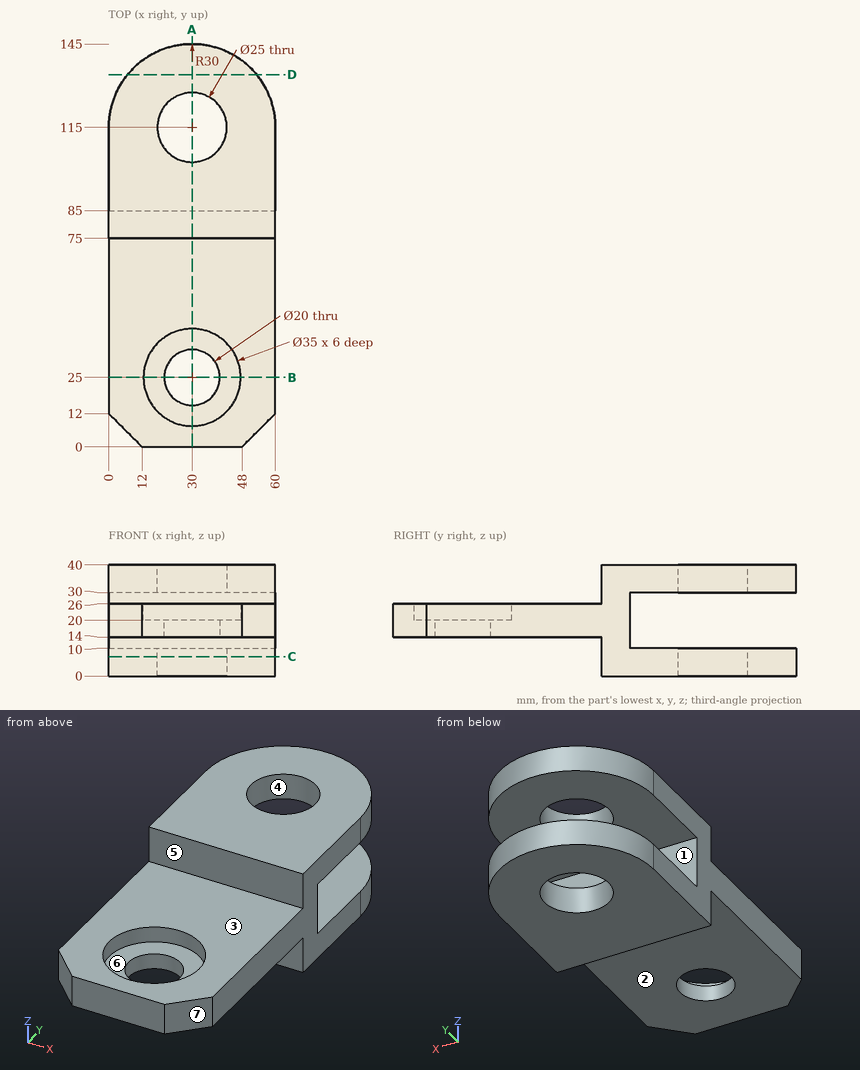
Design review of the part shown in the three views and the two pictorial views. Dimensions are in mm from the part's minimum x, y and z. A direction names the side the tool comes from. Give positions to 0.01 mm unless a question says otherwise; leave off trailing zeros. Loops run counter-clockwise (first coordinate to the right, second up) from the corner with the lowest first, then second, coordinate; pieces in that order, holes last. Notation, with made-up numbers: (19.5, 67) - (44.5, 67) arc R17 cw to (44.5, 79) - close; hole circle Ø9 at (-6, -9.5). An arc over 180 degrees is marked (long way). Use CSV: the item, a comma, the result in double quotes. Start each with the question number.
1. Wall thickness on L1, parallel to Z at x = 15, y = 127; L2, parallel to Y at x = 30, z = 7.75; L3, parallel to Y at x = 30, z = 18.6: over which ranges is each line inside the solid? List them lowest first.
2. Add section A-A (x = 30). State the section outline as (y, z) points, plus the area to 3 significant figures.
3. Insertion check: P1, Ø18, axis at x = 40.5, y = 52.5, coming from the -Z side; P2, Ø5, axis at y = 114, z = 13.5, coming from the -X side; P3, Ø4, axis at x = 31, z = 13, coming from the +Y side; P4, Ø10, axis at x = 36.5, y = 40, coming from the +Z side. Each pin has a flat end and moves straight along its axis. Give the tip position at first contact, or say it passes through.
4. Add section D-D (y = 134). State the section outline as (x, z) points, plus the area to 3 significant figures.
5. Add section B-B (y = 25). State the section outline as (x, z) points, plus the area to 3 significant figures.
6. Draft analysis for pull direction X (two halves, no side actions). For the marked faces 4, 5, 6 and 7, state which applies: released by +X, released by -X, zero draft, split by the parting line, or undercut.
7. Add section C-C (z = 7). State the section outline as (x, y) points, plus the area to 3 significant figures.
8. Machinability: for the marked faces 1, 2 and 3, which of the approach directions +Z, -Z, +X, -X, +Y, -Y give a long, thin tool a straight path to every point of the face, cutting with its end or side? Answer none if there is none.
Results found:
1,L1,"z = 0 to 10, 30 to 40"
1,L2,"y = 75 to 102.5, 127.5 to 145"
1,L3,"y = 0 to 15, 35 to 85"
2,outline,"(0, 14) - (15, 14) - (15, 20) - (7.5, 20) - (7.5, 26) - (0, 26) - close; (35, 14) - (75, 14) - (75, 0) - (102.5, 0) - (102.5, 10) - (85, 10) - (85, 30) - (102.5, 30) - (102.5, 40) - (75, 40) - (75, 26) - (42.5, 26) - (42.5, 20) - (35, 20) - close; (127.5, 0) - (145, 0) - (145, 10) - (127.5, 10) - close; (127.5, 30) - (145, 30) - (145, 40) - (127.5, 40) - close"
2,area,"1,670 mm²"
3,P1,"stops at z = 14"
3,P2,"passes through"
3,P3,"stops at y = 85"
3,P4,"stops at z = 26"
4,outline,"(6.78, 0) - (53.22, 0) - (53.22, 10) - (6.78, 10) - close; (6.78, 30) - (53.22, 30) - (53.22, 40) - (6.78, 40) - close"
4,area,"929 mm²"
5,outline,"(0, 14) - (20, 14) - (20, 20) - (12.5, 20) - (12.5, 26) - (0, 26) - close; (40, 14) - (60, 14) - (60, 26) - (47.5, 26) - (47.5, 20) - (40, 20) - close"
5,area,"390 mm²"
6,face 4,"undercut"
6,face 5,"zero draft"
6,face 6,"undercut"
6,face 7,"released by +X"
7,outline,"(0, 75) - (60, 75) - (60, 115) arc R30 ccw to (0, 115) - close; hole circle Ø25 at (30, 115)"
7,area,"3,320 mm²"
8,face 1,"+X, -X, +Y"
8,face 2,"-Z, +X, -X, -Y"
8,face 3,"+Z, +X, -X, -Y"
